Design review of the part built by this model. Coordinates are the model's own, in mm. Face numbers are marked on the shaded views. A direction names the side the tool comes from. Give positions to 0.01 mm unless a question says otherwise; leave off trailing zeros. Order: outer loops, then holes, each group sorted by start corner. A loop starts at its lowest first (then second) coordinate and runs counter-clockwise, first axis right, second up. Notation, with made-up numbers: M -23,-32.75 L -18,-32.75 A19 ccw -18,-1.75 Z; hole C -25.5,-1.5 d5. An arc over 180 degrees is marked long. Answer as a JSON object with one key per item and string values.
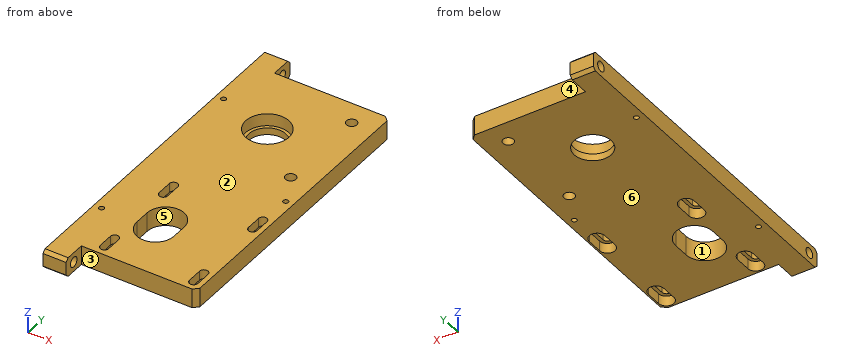
from build123d import *

# Parameters (mm, degrees)
SKETCH_1_W               = 90
SKETCH_1_H               = 220
EXTRUDE_1_DEPTH          = 12.5
SKETCH_2_R               = 12
CUT_EXTRUDE_1_DEPTH      = 239.025733903
HOLE_WIZARD_1_AT_2_COUNT = 2
HOLE_WIZARD_1_AT_2_PITCH = 57.982756057
HOLE_WIZARD_1_AT_3_COUNT = 2
HOLE_WIZARD_1_AT_3_PITCH = 82
HOLE_WIZARD_1_AT_4_COUNT = 2
HOLE_WIZARD_1_AT_4_PITCH = 57.982756057
HOLE_WIZARD_M4_1_D       = 3.3
CUT_EXTRUDE_5_DEPTH      = 239.025733903
CUT_EXTRUDE_6_DEPTH      = 6.5
SKETCH_14_R              = 12
CUT_EXTRUDE_7_DEPTH      = 239.025733903
SKETCH_15_R              = 14
CUT_EXTRUDE_8_DEPTH      = 8
HOLE_WIZARD_M8_1_D       = 6.8
SKETCH_19_W              = 12.5
SKETCH_19_H              = 15
CUT_EXTRUDE_10_DEPTH     = 75
CHAMFER_1_SIZE           = 2
CHAMFER_2_SIZE           = 3
SKETCH_20_R              = 3.25
CUT_EXTRUDE_11_DEPTH     = 233.76866198


with BuildPart() as part:
    # 草图1 → 凸台-拉伸1 (new body)
    with BuildSketch(Plane.XY):
        with Locations((-45, 110)):
            Rectangle(SKETCH_1_W, SKETCH_1_H)
    extrude(amount=EXTRUDE_1_DEPTH)

    # 草图2 → 切除-拉伸1 (cut, through all)
    with BuildSketch(Plane.XY.offset(12.5)):
        with Locations((-50, 55)):
            Circle(SKETCH_2_R)
    extrude(amount=-CUT_EXTRUDE_1_DEPTH, mode=Mode.SUBTRACT)

    # 草图3 → 打孔尺寸根据内六角圆柱头螺钉的类型1 (revolve, cut)
    with BuildSketch(Plane(origin=(-6.008621971, 83.991378029, 12.5), x_dir=(0, -1, 0), z_dir=(1, 0, 0))):
        Polygon((0, 0), (0, 12.5), (5, 12.5), (5, 6), (2.75, 6), (2.75, 0), align=None)
    hole_wizard_1 = revolve(axis=Axis((-6.008621971, 83.991378029, 18.85), (0, 0, -1)), mode=Mode.SUBTRACT)

    # 打孔尺寸根据内六角圆柱头螺钉的类型1 at 2: 打孔尺寸根据内六角圆柱头螺钉的类型1 ×2
    with Locations(*[(0, -i * HOLE_WIZARD_1_AT_2_PITCH, 0) for i in range(1, HOLE_WIZARD_1_AT_2_COUNT)]):
        add(hole_wizard_1, mode=Mode.SUBTRACT)

    # 打孔尺寸根据内六角圆柱头螺钉的类型1 at 3: 打孔尺寸根据内六角圆柱头螺钉的类型1 ×2
    with Locations(*[Vector(-0.7071067811865412, -0.7071067811865539, 0) * (i * HOLE_WIZARD_1_AT_3_PITCH) for i in range(1, HOLE_WIZARD_1_AT_3_COUNT)]):
        add(hole_wizard_1, mode=Mode.SUBTRACT)

    # 打孔尺寸根据内六角圆柱头螺钉的类型1 at 4: 打孔尺寸根据内六角圆柱头螺钉的类型1 ×2
    with Locations(*[(-i * HOLE_WIZARD_1_AT_4_PITCH, 0, 0) for i in range(1, HOLE_WIZARD_1_AT_4_COUNT)]):
        add(hole_wizard_1, mode=Mode.SUBTRACT)

    # M4 螺纹孔1 (through all)
    with Locations(Plane.XY.offset(12.5)):
        with Locations((-85, 170), (-85, 50), (-5, 110)):
            Hole(HOLE_WIZARD_M4_1_D / 2)

    # 草图12 → 切除-拉伸5 (cut, through all)
    with BuildSketch(Plane(origin=(0, 0, 0), x_dir=(-1, 0, 0), z_dir=(0, 0, -1))):
        with BuildLine():
            Line((38, 50), (38, 60))
            ThreePointArc((38, 60), (50, 72), (62, 60))
            Line((62, 60), (62, 50))
            ThreePointArc((62, 50), (50, 38), (38, 50))
        make_face()
        with BuildLine():
            Line((61.241378029, 78.991378029), (61.241378029, 88.991378029))
            ThreePointArc((61.241378029, 88.991378029), (63.991378029, 91.741378029), (66.741378029, 88.991378029))
            Line((66.741378029, 88.991378029), (66.741378029, 78.991378029))
            ThreePointArc((66.741378029, 78.991378029), (63.991378029, 76.241378029), (61.241378029, 78.991378029))
        make_face()
        with BuildLine():
            Line((66.741378029, 31.008621971), (66.741378029, 21.008621971))
            ThreePointArc((66.741378029, 21.008621971), (63.991378029, 18.258621971), (61.241378029, 21.008621971))
            Line((61.241378029, 21.008621971), (61.241378029, 31.008621971))
            ThreePointArc((61.241378029, 31.008621971), (63.991378029, 33.758621971), (66.741378029, 31.008621971))
        make_face()
        with BuildLine():
            Line((8.758621971, 31.008621971), (8.758621971, 21.008621971))
            ThreePointArc((8.758621971, 21.008621971), (6.008621971, 18.258621971), (3.258621971, 21.008621971))
            Line((3.258621971, 21.008621971), (3.258621971, 31.008621971))
            ThreePointArc((3.258621971, 31.008621971), (6.008621971, 33.758621971), (8.758621971, 31.008621971))
        make_face()
        with BuildLine():
            Line((8.758621971, 88.991378029), (8.758621971, 78.991378029))
            ThreePointArc((8.758621971, 78.991378029), (6.008621971, 76.241378029), (3.258621971, 78.991378029))
            Line((3.258621971, 78.991378029), (3.258621971, 88.991378029))
            ThreePointArc((3.258621971, 88.991378029), (6.008621971, 91.741378029), (8.758621971, 88.991378029))
        make_face()
    extrude(amount=-CUT_EXTRUDE_5_DEPTH, mode=Mode.SUBTRACT)

    # 草图13 → 切除-拉伸6 (cut)
    with BuildSketch(Plane(origin=(0, 0, 0), x_dir=(-1, 0, 0), z_dir=(0, 0, -1))):
        with BuildLine():
            Line((11.008621971, 88.991378029), (11.008621971, 78.991378029))
            ThreePointArc((11.008621971, 78.991378029), (6.008621971, 73.991378029), (1.008621971, 78.991378029))
            Line((1.008621971, 78.991378029), (1.008621971, 88.991378029))
            ThreePointArc((1.008621971, 88.991378029), (6.008621971, 93.991378029), (11.008621971, 88.991378029))
        make_face()
        with BuildLine():
            Line((68.991378029, 88.991378029), (68.991378029, 78.991378029))
            ThreePointArc((68.991378029, 78.991378029), (63.991378029, 73.991378029), (58.991378029, 78.991378029))
            Line((58.991378029, 78.991378029), (58.991378029, 88.991378029))
            ThreePointArc((58.991378029, 88.991378029), (63.991378029, 93.991378029), (68.991378029, 88.991378029))
        make_face()
        with BuildLine():
            Line((11.008621971, 31.008621971), (11.008621971, 21.008621971))
            ThreePointArc((11.008621971, 21.008621971), (6.008621971, 16.008621971), (1.008621971, 21.008621971))
            Line((1.008621971, 21.008621971), (1.008621971, 31.008621971))
            ThreePointArc((1.008621971, 31.008621971), (6.008621971, 36.008621971), (11.008621971, 31.008621971))
        make_face()
        with BuildLine():
            Line((68.991378029, 31.008621971), (68.991378029, 21.008621971))
            ThreePointArc((68.991378029, 21.008621971), (63.991378029, 16.008621971), (58.991378029, 21.008621971))
            Line((58.991378029, 21.008621971), (58.991378029, 31.008621971))
            ThreePointArc((58.991378029, 31.008621971), (63.991378029, 36.008621971), (68.991378029, 31.008621971))
        make_face()
    extrude(amount=-CUT_EXTRUDE_6_DEPTH, mode=Mode.SUBTRACT)

    # 草图14 → 切除-拉伸7 (cut, through all)
    with BuildSketch(Plane(origin=(0, 0, 0), x_dir=(-1, 0, 0), z_dir=(0, 0, -1))):
        with Locations((50, 160)):
            Circle(SKETCH_14_R)
    extrude(amount=-CUT_EXTRUDE_7_DEPTH, mode=Mode.SUBTRACT)

    # 草图15 → 切除-拉伸8 (cut)
    with BuildSketch(Plane.XY.offset(12.5)):
        with Locations((-50, 160)):
            Circle(SKETCH_15_R)
    extrude(amount=-CUT_EXTRUDE_8_DEPTH, mode=Mode.SUBTRACT)

    # M8 螺纹孔1 (through all)
    with Locations(Plane.XY.offset(12.5)):
        with Locations((-15, 130), (-15, 190)):
            Hole(HOLE_WIZARD_M8_1_D / 2)

    # 草图19 → 切除-拉伸10 (cut)
    with BuildSketch(Plane(origin=(0, 0, 0), x_dir=(0, 0, -1), z_dir=(1, 0, 0))):
        with Locations((-6.25, 212.5)):
            Rectangle(SKETCH_19_W, SKETCH_19_H)
        with Locations((-6.25, 7.5)):
            Rectangle(SKETCH_19_W, SKETCH_19_H)
    extrude(amount=-CUT_EXTRUDE_10_DEPTH, mode=Mode.SUBTRACT)

    # 倒角1
    chamfer_1_edges = [part.edges().sort_by_distance(p)[0] for p in [
        (-82.5, 220, 0),
        (-82.5, 220, 12.5),
        (-82.5, 0, 0),
        (-82.5, 0, 12.5),
    ]]
    chamfer(chamfer_1_edges, length=CHAMFER_1_SIZE)

    # 倒角2
    chamfer_2_edges = [part.edges().sort_by_distance(p)[0] for p in [
        (0, 205, 6.25),
        (0, 15, 6.25),
    ]]
    chamfer(chamfer_2_edges, length=CHAMFER_2_SIZE)

    # 草图20 → 切除-拉伸11 (cut, through all)
    with BuildSketch(Plane(origin=(-75, 0, 0), x_dir=(0, 0, -1), z_dir=(1, 0, 0))):
        with Locations((-6.25, 212.5)):
            Circle(SKETCH_20_R)
        with Locations(Location((-6.25, 7.5, 0), (0, 0, 180))):
            Circle(SKETCH_20_R)
    extrude(amount=-CUT_EXTRUDE_11_DEPTH, mode=Mode.SUBTRACT)


solid = part.part
(1) We need section D-D (x = -15). Write out the cut boundary in (y, z), plus the area to 4 significant figures.
Checked values:
{"outline": "M 15,0 L 126.6,0 L 126.6,12.5 L 15,12.5 Z; M 133.4,0 L 186.6,0 L 186.6,12.5 L 133.4,12.5 Z; M 193.4,0 L 205,0 L 205,12.5 L 193.4,12.5 Z", "area": "2,205 mm^2"}
(2) Insertion check: pin 1 (7.5 mm diameter, centred on y = 7.5, z = 6.25, fed in from +X); pin 2 (1.5 mm diameter, centred on x = -65.5, z = 9.5, fed in from -Y); pin 3 (4.5 mm diameter, centred on x = -85, y = 170, fed in from +Z); pin 4 (2.5 mm diameter, centred on x = -85, y = 50, fed in from -Z). Each pin has a flat end and moves straight along its axis. Give the tip position at first contact, or say it passes through.
Checked values:
{"pin 1": "stops at x = -75", "pin 2": "stops at y = 15", "pin 3": "stops at z = 12.5", "pin 4": "passes through"}
(3) Tool access review of the marked faces 1, 2 and 3: name each direction out of +Z, -Z, +X, -X, +Y, -Y from which nothing blocks a thin tool from reaching the whole face with its end or side.
Checked values:
{"face 1": "+Z, -Z", "face 2": "+Z, +X, -X, +Y, -Y", "face 3": "+Z, -Z, +X, -Y"}
(4) We need section C-C (x = -78.5). Write out the cut boundary in (y, z).
Checked values:
{"outline": "M 0,2 L 2,0 L 218,0 L 220,2 L 220,10.5 L 218,12.5 L 2,12.5 L 0,10.5 Z; hole C 7.5,6.25 d6.5; hole C 212.5,6.25 d6.5"}
(5) To check wall thickness, follow L1, parallel to Y at x = -50, z = 11; L2, parallel to X at y = 190, z = 10; L3, parallel to Y at x = -8, z = 1. State the ranges of each line that lie inside material, in increasing order. Write a range as from..to.
Checked values:
{"L1": "y = 15..38, 72..146, 174..205", "L2": "x = -90..-18.4, -11.6..0", "L3": "y = 15..16.42, 35.59..74.41, 93.58..205"}
(6) We need section A-A (x = -50). Write out the cut boundary in (y, z), plus the area to 3 significant figures.
Checked values:
{"outline": "M 15,0 L 38,0 L 38,12.5 L 15,12.5 Z; M 72,0 L 148,0 L 148,4.5 L 146,4.5 L 146,12.5 L 72,12.5 Z; M 172,0 L 205,0 L 205,12.5 L 174,12.5 L 174,4.5 L 172,4.5 Z", "area": "1,620 mm^2"}
(7) We need section B-B (y = 212.5). Write out the cut boundary in (x, z), plus the area to 3 significant figures.
Checked values:
{"outline": "M -90,0 L -75,0 L -75,3 L -90,3 Z; M -90,9.5 L -75,9.5 L -75,12.5 L -90,12.5 Z", "area": "90.0 mm^2"}
(8) Draft analysis for pull direction Y (two halves, no side actions). For the marked faces 4, 5 and 6, state which applies: +Y half, -Y half, draft (parallel to the pull), parting line (faces both ways), or undercut.
Checked values:
{"face 4": "+Y half", "face 5": "undercut", "face 6": "draft"}
